from build123d import *

# Parameters (mm, degrees)
BOSS_EXTRUDE1_DEPTH = 5


with BuildPart() as part:
    # Sketch1 → Boss-Extrude1 (new body)
    with BuildSketch(Plane(origin=(0, 0, 0), x_dir=(1, 0, 0), z_dir=(0, 1, 0))):
        with BuildLine():
            Line((-348.959440129, 10), (26.040559871, 10))
            ThreePointArc((26.040559871, 10), (36.040559871, 0), (26.040559871, -10))
            Line((26.040559871, -10), (-348.959440129, -10))
            ThreePointArc((-348.959440129, -10), (-358.959440129, 0), (-348.959440129, 10))
        make_face()
        with BuildLine():
            Line((-348.959440129, 8), (26.040559871, 8))
            ThreePointArc((26.040559871, 8), (34.040559871, 0), (26.040559871, -8))
            Line((26.040559871, -8), (-348.959440129, -8))
            ThreePointArc((-348.959440129, -8), (-356.959440129, 0), (-348.959440129, 8))
        make_face(mode=Mode.SUBTRACT)
    extrude(amount=BOSS_EXTRUDE1_DEPTH)


solid = part.part
Check sheet for the modelled part. Datum: model origin and axes. Units: mm. A direction names the side the tool comes from. Coordinates: 2 decimals unless noted, no trailing zeros. Write each loop counter-clockwise with the first axis right and the second up, starting at its lowest first coordinate (ties: lowest second). Pieces come first, ordered by that corner, then holes. Notation, with made-up numbers: M 11.5,40.5 L 68.5,40.5 A12 cw 68.5,52.5 Z; hole C 49.25,9.5 d11. An arc over 180 degrees is marked long. Answer as CSV lines item,"result".
Q1. Material ranges on probe 1 along Z at (x, y) = (-301, 1.7); probe 2 along X at (y, z) = (3.7, -1); probe 3 along X at (y, z) = (4.25, -2.75) (3 decimals), recorded low to high. Write a range as from..to.
Check result:
probe 1,"-10..-8, 8..10"
probe 2,"-358.91..-356.9, 33.98..35.99"
probe 3,"-358.574..-356.472, 33.553..35.655"
Q2. Go/stop test with flat-tipped pins: pin 1 (3 mm diameter, centred on y = 4.5, z = -7.5, fed in from -X); pin 2 (2 mm diameter, centred on y = 1.5, z = 4.5, fed in from -X). Record where each tip stops, or that it passes through.
Check result:
pin 1,"x = -356.96"
pin 2,"x = -358.33"
Q3. Cross-section at B-B (x = -188.5). Record the boundary of the cut face in (y, z), then the cut area to 3 significant figures.
Check result:
outline,"M 0,-10 L 5,-10 L 5,-8 L 0,-8 Z; M 0,8 L 5,8 L 5,10 L 0,10 Z"
area,"20.0 mm^2"
Q4. Cross-section at A-A (y = 1.45). Record the boundary of the cut face in (x, z).
Check result:
outline,"M -348.96,-10 L 26.04,-10 A10 ccw 26.04,10 L -348.96,10 A10 ccw Z; hole M -348.96,-8 L 26.04,-8 A8 ccw 26.04,8 L -348.96,8 A8 ccw Z"
Q5. Cross-section at C-C (z = 0). Record the boundary of the cut face in (x, y), then the cut area to 3 significant figures.
Check result:
outline,"M -358.96,0 L -356.96,0 L -356.96,5 L -358.96,5 Z; M 34.04,0 L 36.04,0 L 36.04,5 L 34.04,5 Z"
area,"20.0 mm^2"
Q6. Mould release check, pull along X, two halves, no side actions. Record for faces 1 (the face through (-356.958, 2.465, 0.176)), 2 (the face through (36.04, 2.46, -0.22)), 3 (the face through (-160.5, 5, -8.2)): released by +X, released by -X, zero draft, split by the parting line, or undercut.
Check result:
face 1,"undercut"
face 2,"released by +X"
face 3,"zero draft"
Q7. Set-up check for faces 4 (the face through (34.04, 2.46, -0.18)), 5 (the face through (-160.5, 0, -8.2)): record each of +Z, -Z, +X, -X, +Y, -Y from which the full face is reachable in a straight line by a thin tool's end or side.
Check result:
face 4,"+Y, -Y"
face 5,"+Z, -Z, +X, -X, -Y"
